Geometry: final body of the model. Coordinates: model frame, mm. A direction names the side the tool comes from. Give positions to 0.01 mm unless a question says otherwise; leave off trailing zeros. Write each loop counter-clockwise with the first axis right and the second up, starting at its lowest first coordinate (ties: lowest second). Pieces come first, ordered by that corner, then holes. Notation, with made-up numbers: (-6, -12) - (34, -12) arc R14 ccw to (34, -3) - close; hole circle Ø8 at (85.25, 53.25). An arc over 180 degrees is marked (long way). Use CSV: the item, a comma, the result in double quotes. Start each with the question number.
(1) Section D-D on y = 10.5. Output: boundary loops of the cut face in (x, z), and give its area (3 significant figures).
(2) Reachability of faces 4 (the flat face through (0, 11, -30.5)), 5 (the cylindrical face through (-19.715, 10.409, -30.801)), 6 (the flat face through (0, 8, -40)), 7 (the cylindrical face through (-14, 2, -4)), 8 (the cylindrical face through (19.715, 10.409, -30.801)) from +Z, -Z, +X, -X, +Y, -Y: full face, straight path, thin tool, end or side. Return the list, or none.
(3) Line query: probe 1 along X at (y, z) = (1.75, -4); probe 2 along Z at (x, y) = (16, 1.75); probe 3 along Z at (x, y) = (-14.5, 1.75). Output: solid intervals per line, ascending. Write a range as [from, to].
(4) Section B-B on y = 4.75. Output: boundary loops of the cut face in (x, z), and give its area (3 significant figures).
(5) Section A-A on z = -36. Output: boundary loops of the cut face in (x, y).
(6) Section C-C on x = 0. Output: boundary loops of the cut face in (y, z).
(7) Draft query along X for faces 1 (the cylindrical face through (-17.774, 8.381, -35.077)), 2 (the flat face through (0, 4, -9)), 3 (the cylindrical face through (-19.715, 1.972, -0.301)). Return one class per face: released by +X, released by -X, zero draft, split by the parting line, or undercut.
(8) First-contact query: pin 1 Ø16 at (x, z) = (-9.5, -14.5) entering from +Y; pin 2 Ø5 at (x, z) = (16, -36) entering from +Y. Flat tips, straight axial feed; report the tip coordinate or a pass-through.
from build123d import *

# Parameters (mm, degrees)
BOSS_EXTRUDE1_DEPTH     = 20
CUT_EXTRUDE1_DEPTH      = 47.572524089
CUT_EXTRUDE1_DEPTH_BACK = 47.572524089
SKETCH2_R               = 10
SKETCH2_R_2             = 2
FILLET1_R               = 1
SKETCH3_R               = 3
SKETCH3_R_2             = 1.25
CUT_EXTRUDE2_DEPTH      = 41.239905566


with BuildPart() as part:
    # Sketch1 → Boss-Extrude1 (new, symmetric)
    with BuildSketch(Plane(origin=(0, 0, 0), x_dir=(0, 0, -1), z_dir=(1, 0, 0))):
        Polygon((0, 0), (40, 0), (40, 4), (40, 17), (30.5, 17), (30.5, 4), (0, 4), align=None)
    extrude(amount=BOSS_EXTRUDE1_DEPTH, both=True)

    # Sketch2 → Cut-Extrude1 (cut, two sides: drawn at the far end of the back side and taken through both)
    with BuildSketch(Plane(origin=(0, 4, 0), x_dir=(1, 0, 0), z_dir=(0, 1, 0)).offset(-CUT_EXTRUDE1_DEPTH_BACK)):
        with Locations(Location((0, 20, 0), (0, 0, 270))):
            Circle(SKETCH2_R)
        with Locations(Location((16, 36, 0), (0, 0, 270))):
            Circle(SKETCH2_R_2)
        with Locations(Location((16, 4, 0), (0, 0, 270))):
            Circle(SKETCH2_R_2)
        with Locations(Location((-16, 4, 0), (0, 0, 270))):
            Circle(SKETCH2_R_2)
        with Locations(Location((-16, 36, 0), (0, 0, 270))):
            Circle(SKETCH2_R_2)
    extrude(amount=CUT_EXTRUDE1_DEPTH + CUT_EXTRUDE1_DEPTH_BACK, mode=Mode.SUBTRACT)

    # Fillet1
    fillet1_edges = [part.edges().sort_by_distance(p)[0] for p in [
        (20, 8.5, -40),
        (20, 10.5, -30.5),
        (20, 2, 0),
        (-20, 10.5, -30.5),
        (-20, 8.5, -40),
        (-20, 2, 0),
    ]]
    fillet(fillet1_edges, radius=FILLET1_R)

    # Sketch3 → Cut-Extrude2 (cut, through all)
    with BuildSketch(Plane.XY.offset(-30.5)):
        with Locations((5.5, 11)):
            Circle(SKETCH3_R)
        with Locations((-15, 10.5)):
            Circle(SKETCH3_R_2)
    extrude(amount=-CUT_EXTRUDE2_DEPTH, mode=Mode.SUBTRACT)


solid = part.part
Check values:
1,outline,"(-20, -39) arc R1 ccw to (-19, -40) - (-16.25, -40) - (-16.25, -37.98) arc R2 cw to (-16.25, -34.02) - (-16.25, -30.5) - (-19, -30.5) arc R1 ccw to (-20, -31.5) - close; (-13.75, -40) - (2.54, -40) - (2.54, -30.5) - (-13.75, -30.5) - close; (8.46, -40) - (19, -40) arc R1 ccw to (20, -39) - (20, -31.5) arc R1 ccw to (19, -30.5) - (8.46, -30.5) - close; hole circle Ø4 at (16, -36)"
1,area,"281 mm²"
2,face 4,"+Z, +X, -X, +Y"
2,face 5,"+Z, -X, +Y"
2,face 6,"-Z, +X, -X, +Y, -Y"
2,face 7,"+Y, -Y"
2,face 8,"+Z, +X, +Y"
3,probe 1,"x = [-20, -18], [-14, 14], [18, 20]"
3,probe 2,"z = [-40, -38], [-34, -6], [-2, 0]"
3,probe 3,"z = [-40, -37.32], [-34.68, -5.32], [-2.68, 0]"
4,outline,"(-20, -39) arc R1 ccw to (-19, -40) - (19, -40) arc R1 ccw to (20, -39) - (20, -31.5) arc R1 ccw to (19, -30.5) - (-19, -30.5) arc R1 ccw to (-20, -31.5) - close; hole circle Ø4 at (-16, -36); hole circle Ø4 at (16, -36)"
4,area,"354 mm²"
5,outline,"(-20, 0) - (-18, 0) - (-18, 17) - (-20, 17) - close; (-14, 0) - (14, 0) - (14, 17) - (-14, 17) - (-14, 11.25) arc R1.25 cw to (-14, 9.75) - close; (18, 0) - (20, 0) - (20, 17) - (18, 17) - close; hole circle Ø6 at (5.5, 11)"
6,outline,"(0, -40) - (17, -40) - (17, -30.5) - (4, -30.5) - (4, -30) - (0, -30) - close; (0, -10) - (4, -10) - (4, 0) - (0, 0) - close"
7,face 1,"undercut"
7,face 2,"zero draft"
7,face 3,"released by -X"
8,pin 1,"stops at y = 4"
8,pin 2,"stops at y = 17"
